For this review, take the finished solid that the model builds, in its own axes (mm). Give positions to 0.01 mm unless a question says otherwise; leave off trailing zeros. Write each loop counter-clockwise with the first axis right and the second up, starting at its lowest first coordinate (ties: lowest second). Pieces come first, ordered by that corner, then holes.
1) We need section A-A on x = 10.56. Give the boundary of the cut face in (y, z).
2) For P1, Ø3.5, axis at x = -45, y = -32.5, coming from the -Z side, flat-tipped, find the tip position at first contact; note if it passes through.
3) We need section B-B on y = -32.5. Give the boundary of the cut face in (x, z).
4) Wall thickness on line 1 along Y through (x, z) = (43.86, 0.6); line 2 along X through (y, z) = (-30, -0.25); line 3 along Y through (x, z) = (-43.86, 1.25): over which ranges is each line inside the solid? List them lowest first.
5) We need section D-D on x = 43.86. Give the boundary of the cut face in (y, z).
6) We need section C-C on z = -1.3. Give the number of separate pieces and of enclosed holes in the cut face, and give its area (3 significant figures).
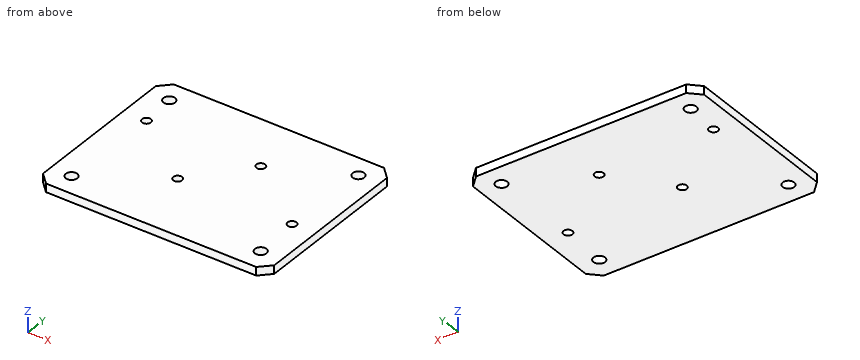
from build123d import *

# Parameters (mm, degrees)
SKETCH_1_W                  = 110
SKETCH_1_H                  = 85
EXTRUDE_1_DEPTH             = 2
CHAMFER_1_SIZE              = 5
HOLE_WIZARD_5_5_5_5_1_D     = 5.5
HOLE_WIZARD_5_5_5_5_1_DEPTH = 15.61
HOLE_WIZARD_5_5_5_5_1_TIP   = 1.58771324
HOLE_WIZARD_M5_3_D          = 4.2


with BuildPart() as part:
    # 草图1 → 凸台-拉伸1 (new, symmetric)
    with BuildSketch(Plane.XY):
        Rectangle(SKETCH_1_W, SKETCH_1_H)
    extrude(amount=EXTRUDE_1_DEPTH, both=True)

    # 倒角1
    chamfer_1_edges = [part.edges().sort_by_distance(p)[0] for p in [
        (-55, 42.5, 0),
        (55, 42.5, 0),
        (55, -42.5, 0),
        (-55, -42.5, 0),
    ]]
    chamfer(chamfer_1_edges, length=CHAMFER_1_SIZE)

    # Ø5.5 (5.5) 直径孔1
    with Locations(Plane.XY.offset(2)):
        with Locations((45, 32.5), (45, -32.5), (-45, -32.5), (-45, 32.5)):
            Hole(HOLE_WIZARD_5_5_5_5_1_D / 2, depth=HOLE_WIZARD_5_5_5_5_1_DEPTH)
            with Locations((0, 0, -(HOLE_WIZARD_5_5_5_5_1_DEPTH + HOLE_WIZARD_5_5_5_5_1_TIP / 2))):  # 120° drill point
                Cone(0, HOLE_WIZARD_5_5_5_5_1_D / 2, HOLE_WIZARD_5_5_5_5_1_TIP, mode=Mode.SUBTRACT)

    # M5 螺纹孔3 (through all)
    with Locations(Plane.XY.offset(2)):
        with Locations((-43.86, 15.732567746), (10.56, 15.732567746), (-10.56, -10.077432254), (43.86, -10.077432254)):
            Hole(HOLE_WIZARD_M5_3_D / 2)


solid = part.part
Results list:
1. outline: (-42.5, -2) - (13.63, -2) - (13.63, 2) - (-42.5, 2) - close; (17.83, -2) - (42.5, -2) - (42.5, 2) - (17.83, 2) - close
2. P1: passes through
3. outline: (-55, -2) - (-47.75, -2) - (-47.75, 2) - (-55, 2) - close; (-42.25, -2) - (42.25, -2) - (42.25, 2) - (-42.25, 2) - close; (47.75, -2) - (55, -2) - (55, 2) - (47.75, 2) - close
4. line 1: y = -42.5 to -35, -30 to -12.18, -7.98 to 30, 35 to 42.5
4. line 2: x = -55 to -46.15, -43.85 to 43.85, 46.15 to 55
4. line 3: y = -42.5 to -35, -30 to 13.63, 17.83 to 30, 35 to 42.5
5. outline: (-42.5, -2) - (-35, -2) - (-35, 2) - (-42.5, 2) - close; (-30, -2) - (-12.18, -2) - (-12.18, 2) - (-30, 2) - close; (-7.98, -2) - (30, -2) - (30, 2) - (-7.98, 2) - close; (35, -2) - (42.5, -2) - (42.5, 2) - (35, 2) - close
6. separate pieces: 1
6. enclosed holes: 8
6. area: 9,150 mm2
